Here's how the part is built. I have some questions about the finished solid (model axes, mm). A direction names the side the tool comes from. Give positions to 0.01 mm unless a question says otherwise; leave off trailing zeros. Write each loop counter-clockwise with the first axis right and the second up, starting at its lowest first coordinate (ties: lowest second). Pieces come first, ordered by that corner, then holes. Notation, with made-up numbers: (-38, 22) -> (0, 22) arc R10 cw to (0, 31) -> close; hole circle Ø3 at (43, 59). An arc over 180 degrees is marked (long way). Use CSV: the item, a comma, the result in double quotes. Start each with the question number.
(1) If we mould it in two halves opening along Z, with no side actions, what happens to faces 5 (the flat face through (0, 0, -11)), 6 (the cylindrical face through (-3.18, 33.78, -0.27)), 7 (the cylindrical face through (-5.857, 19.72, -1.301))? For each: pulls with the +Z half, pulls with the -Z half, needs draft (parallel to the pull), parting line crosses it, or undercut.
(2) Suppose I cut it at C-C on z = 10. List the corners of the cut face in (x, y) for me, plus the area to 3 significant figures.
(3) Suppose I cut it at A-A on z = 0. List the corners of the cut face in (x, y) for me (3 decimals).
(4) I need wall thicknesses on L1, parallel to Y at x = -3.35, z = 0; L2, parallel to Y at x = 0.5, z = 0.5; L3, parallel to Y at x = 3.5, z = 4. Which ranges of each line are inside material? Lowest first, please. Write a range as [from, to].
(5) Which directions (+Z, -Z, +X, -X, +Y, -Y) give clear straight access to the entire face, cutting with the end or side of a thin tool? Please do faces 1 (the flat face through (-2.5, -49, 0)), 2 (the cylindrical face through (0, -49, -16)), 3 (the flat face through (0, 33, 0)), 4 (the flat face through (2.5, -49, 0)).
(6) Suppose I cut it at B-B on y = 35. List the corners of the cut face in (x, z) for me (3 decimals).
(7) For pin 1 Ø5 at (y, z) = (-42, -7.5) entering from +X; pin 2 Ø1.1 at (x, z) = (-3.5, 2) entering from -Y; pin 3 Ø3 at (x, z) = (0, 8) entering from +Y, each with a flat end and sliding along its axis, tell me the tip position at first contact or that it passes through.
(8) Suppose I cut it at D-D on y = 12. List the corners of the cut face in (x, z) for me, plus the area to 3 significant figures.
from build123d import *

# Parameters (mm, degrees)
SKETCH1_R                   = 6
BOSS_EXTRUDE1_DEPTH         = 40
CUT_EXTRUDE1_DEPTH          = 41.890096601
CUT_EXTRUDE1_DEPTH_BACK     = 41.890096601
SKETCH2_W                   = 18.470240229
SKETCH2_H                   = 11
M3_TAPPED_HOLE2_D           = 2.5
M3_TAPPED_HOLE2_CSINK_D     = 3.05
M3_TAPPED_HOLE2_CSINK_ANGLE = 90
SKETCH5_R                   = 16
BOSS_EXTRUDE2_DEPTH         = 100
CUT_EXTRUDE2_DEPTH          = 142.816783309
CUT_EXTRUDE2_DEPTH_BACK     = 100
SKETCH11_OUTSIDE_W          = 63.426
SKETCH11_OUTSIDE_H          = 63.426
SKETCH11_OUTSIDE_W_2        = 5
SKETCH11_OUTSIDE_H_2        = 40.425128238


with BuildPart() as part:
    # Sketch1 → Boss-Extrude1 (new body)
    with BuildSketch(Plane(origin=(0, 0, 0), x_dir=(1, 0, 0), z_dir=(0, 1, 0))):
        with Locations(Location((0, 0, 0), (0, 0, 270))):
            Circle(SKETCH1_R)
    extrude(amount=BOSS_EXTRUDE1_DEPTH)

    # Sketch2 → Cut-Extrude1 (cut, two sides: drawn at the far end of the back side and taken through both)
    with BuildSketch(Plane.XY.offset(-CUT_EXTRUDE1_DEPTH_BACK)):
        with Locations((9.235120115, 34.5)):
            Rectangle(SKETCH2_W, SKETCH2_H)
    extrude(amount=CUT_EXTRUDE1_DEPTH + CUT_EXTRUDE1_DEPTH_BACK, mode=Mode.SUBTRACT)

    # M3 Tapped Hole2 (through all)
    with Locations(Plane(origin=(0, 0, 0), x_dir=(0, 0, -1), z_dir=(1, 0, 0))):
        with Locations((0, 35)):
            CounterSinkHole(M3_TAPPED_HOLE2_D / 2, M3_TAPPED_HOLE2_CSINK_D / 2, counter_sink_angle=M3_TAPPED_HOLE2_CSINK_ANGLE)

    # Sketch5 → Boss-Extrude2 (add)
    with BuildSketch(Plane.XZ):
        with Locations(Location((0, 0, 0), (0, 0, 270))):
            Circle(SKETCH5_R)
    extrude(amount=BOSS_EXTRUDE2_DEPTH)

    # Sketch11 outside → Cut-Extrude2 (cut, two sides: drawn at the far end of the back side and taken through both)
    with BuildSketch(Plane.XZ.offset(100).offset(-CUT_EXTRUDE2_DEPTH_BACK)):
        Rectangle(SKETCH11_OUTSIDE_W, SKETCH11_OUTSIDE_H)
        Rectangle(SKETCH11_OUTSIDE_W_2, SKETCH11_OUTSIDE_H_2, mode=Mode.SUBTRACT)
    extrude(amount=CUT_EXTRUDE2_DEPTH + CUT_EXTRUDE2_DEPTH_BACK, mode=Mode.SUBTRACT)


solid = part.part
Geometry says:
1,face 5,"needs draft"
1,face 6,"undercut"
1,face 7,"parting line crosses it"
2,outline,"(-2.5, -100) -> (2.5, -100) -> (2.5, 0) -> (-2.5, 0) -> close"
2,area,"500 mm²"
3,outline,"(-6, 0) -> (-2.5, 0) -> (-2.5, -100) -> (2.5, -100) -> (2.5, 0) -> (6, 0) -> (6, 29) -> (0, 29) -> (0, 33.475) -> (-0.275, 33.75) -> (-6, 33.75) -> close; (-6, 36.25) -> (-0.275, 36.25) -> (0, 36.525) -> (0, 40) -> (-6, 40) -> close"
4,L1,"[0, 33.75], [36.25, 40]"
4,L2,"[-100, 29]"
4,L3,"[0, 29]"
5,face 1,"+Z, -Z, -X, -Y"
5,face 2,"-Z, +Y, -Y"
5,face 3,"+Z, -Z, +X, +Y"
5,face 4,"+Z, -Z, +X, -Y"
6,outline,"(-5.868, -1.25) arc R6 ccw to (0, -6) -> (0, -1.525) -> (-0.275, -1.25) -> close; (-5.868, 1.25) -> (-0.275, 1.25) -> (0, 1.525) -> (0, 6) arc R6 ccw to start"
7,pin 1,"x = 2.5"
7,pin 2,"y = 0"
7,pin 3,"y = 0"
8,outline,"circle Ø12 at (0, 0)"
8,area,"113 mm²"
